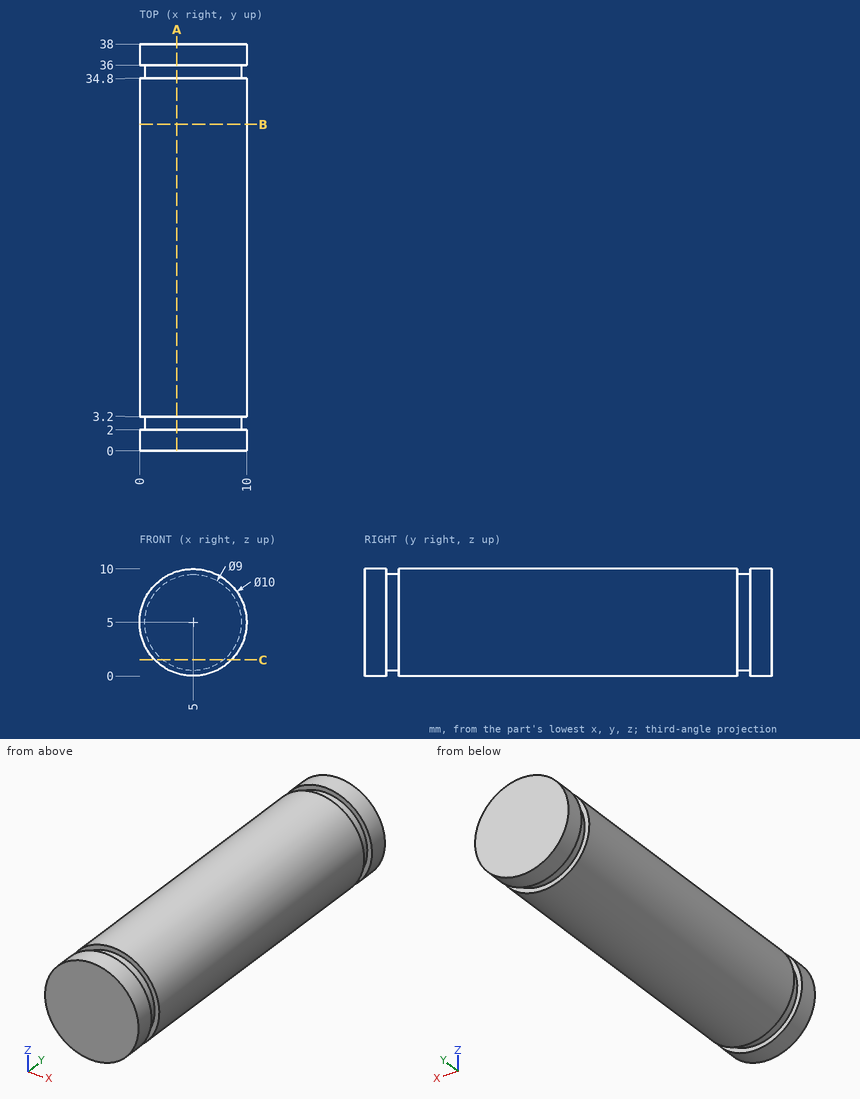
Geometry check sheet. Reference: drawing and pictorial views, mm from the part's lowest x, y, z. Round coordinates to 2 decimals unless told otherwise and drop trailing zeros. Loops run counter-clockwise (first coordinate to the right, second up) from the corner with the lowest first, then second, coordinate; pieces in that order, holes last. Notation, with made-up numbers: M 80,53.25 L 89,53.25 A16 ccw 89,77.25 Z; hole C 67,-8 d11. An arc over 180 degrees is marked long. Return JSON: item names as keys, results as strings. Group by question number.
(1) Section check B-B, the plane y = 30.5. Enter the section's corners in (x, z).
(2) Section check C-C, the plane z = 1.5. Enter the section's corners in (x, y), and give its area (3 significant figures).
(3) Section check A-A, the plane x = 3.5. Enter the section's corners in (y, z), and give its area (3 significant figures).
(4) Go/stop test with a flat-tipped pin: pin 1 (1 mm diameter, centred on y = 13.5, z = 6, fed in from +X). Record where the tip stops, or that it passes through.
(5) Scan lines: line 1 along Y through (x, z) = (0.5, 3.5); line 2 along X through (y, z) = (16.5, 5.25). Record each from-to range of solid material in increasing order. Write a range as [from, to].
Data:
{
 "1": {"outline": "C 5,5 d10"},
 "2": {"outline": "M 1.43,0 L 8.57,0 L 8.57,2 L 7.83,2 L 7.83,3.2 L 8.57,3.2 L 8.57,34.8 L 7.83,34.8 L 7.83,36 L 8.57,36 L 8.57,38 L 1.43,38 L 1.43,36 L 2.17,36 L 2.17,34.8 L 1.43,34.8 L 1.43,3.2 L 2.17,3.2 L 2.17,2 L 1.43,2 Z", "area": "268 mm²"},
 "3": {"outline": "M 0,0.23 L 2,0.23 L 2,0.76 L 3.2,0.76 L 3.2,0.23 L 34.8,0.23 L 34.8,0.76 L 36,0.76 L 36,0.23 L 38,0.23 L 38,9.77 L 36,9.77 L 36,9.24 L 34.8,9.24 L 34.8,9.77 L 3.2,9.77 L 3.2,9.24 L 2,9.24 L 2,9.77 L 0,9.77 Z", "area": "360 mm²"},
 "4": {"pin 1": "x = 9.97"},
 "5": {"line 1": "[0, 2], [3.2, 34.8], [36, 38]", "line 2": "[0.01, 9.99]"}
}
